from build123d import *

# Parameters (mm, degrees)
SKETCH1_R           = 5
BOSS_EXTRUDE1_DEPTH = 25
SKETCH2_R           = 7.5
BOSS_EXTRUDE2_DEPTH = 8
SKETCH3_R           = 5
BOSS_EXTRUDE3_DEPTH = 30
SKETCH4_R           = 7.5
BOSS_EXTRUDE4_DEPTH = 17
CHAMFER1_SIZE       = 1
CHAMFER2_SIZE       = 0.5


with BuildPart() as part:
    # Sketch1 → Boss-Extrude1 (new body)
    with BuildSketch(Plane.XY):
        Circle(SKETCH1_R)
    extrude(amount=BOSS_EXTRUDE1_DEPTH)

    # Sketch2 → Boss-Extrude2 (add)
    with BuildSketch(Plane.XY.offset(25)):
        Circle(SKETCH2_R)
    extrude(amount=BOSS_EXTRUDE2_DEPTH)

    # Sketch3 → Boss-Extrude3 (add)
    with BuildSketch(Plane.XY.offset(33)):
        Circle(SKETCH3_R)
    extrude(amount=BOSS_EXTRUDE3_DEPTH)

    # Sketch4 → Boss-Extrude4 (add)
    with BuildSketch(Plane.XY.offset(33)):
        Circle(SKETCH4_R)
    extrude(amount=BOSS_EXTRUDE4_DEPTH)

    # Chamfer1
    chamfer1_edges = [part.edges().sort_by_distance(p)[0] for p in [
        (-7.5, 0, 50),
    ]]
    chamfer(chamfer1_edges, length=CHAMFER1_SIZE)

    # Chamfer2
    chamfer2_edges = [part.edges().sort_by_distance(p)[0] for p in [
        (-5, 0, 63),
    ]]
    chamfer(chamfer2_edges, length=CHAMFER2_SIZE)


solid = part.part
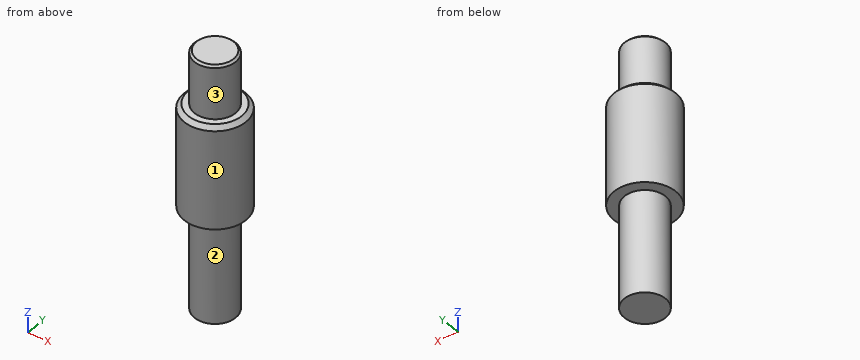
Can you work these out from the model? Positions are in its coordinate system, mm. Face numbers are marked on the shaded views. A direction names the side the tool comes from. Coordinates: 2 decimals unless noted, no trailing zeros. Write each loop counter-clockwise with the first axis right and the second up, starting at its lowest first coordinate (ties: lowest second). Pieces come first, ordered by that corner, then holes. Notation, with made-up numbers: (-39.75, 35.25) -> (-19.75, 35.25) arc R25 ccw to (-19.75, 56.25) -> close; hole circle Ø7 at (85, 18). An arc over 180 degrees is marked (long way). Write each question's results on one line, items separated by ' | '. Start each with the question number.
Item 1: Please list where these lines run through material, in increasing order: probe 1 along Z at (x, y) = (-5.25, -3); probe 2 along X at (y, z) = (5.75, 43); probe 3 along X at (y, z) = (6.5, 33.5).
Item 2: If we section it at D-D, the plane z = 24: Write out the boundary of the cut face in (x, y), and give its area (3 significant figures).
Item 3: I'm going to push flat-ended pins straight in: P1, Ø2, axis at y = 3, z = 19.5, coming from the -X side; P2, Ø6, axis at x = -1, z = 47.5, coming from the -Y side; P3, Ø4, axis at y = 2.5, z = 36.5, coming from the +X side; P4, Ø3, axis at x = 4.5, z = 9, coming from the +Y side. Where does each tip first touch, or does it pass through?
Item 4: If we section it at C-C, the plane z = 34: Write out the boundary of the cut face in (x, y).
Item 5: If we section it at A-A, the plane y = 0: Write out the boundary of the cut face in (x, z), and give its area (3 significant figures).
Item 6: On a 3-axis mill with a long thin cutter (end or side, diameter ignored), from which of +Z, -Z, +X, -X, +Y, -Y can I reach the whole of each face in a straight line? I mean the marked faces 1, 2 and 3. Say none if no direction works.
Answer block:
1) probe 1: 25 to 50 | probe 2: -4.82 to 4.82 | probe 3: -3.74 to 3.74
2) outline: circle Ø10 at (0, 0) | area: 78.5 mm²
3) P1: x = -4.58 | P2: y = -7.5 | P3: x = 7.48 | P4: y = 4
4) outline: circle Ø15 at (0, 0)
5) outline: (-7.5, 25) -> (-5, 25) -> (-5, 0) -> (5, 0) -> (5, 25) -> (7.5, 25) -> (7.5, 49) -> (6.5, 50) -> (5, 50) -> (5, 62.5) -> (4.5, 63) -> (-4.5, 63) -> (-5, 62.5) -> (-5, 50) -> (-6.5, 50) -> (-7.5, 49) -> close | area: 754 mm²
6) face 1: +Z, -Z | face 2: -Z | face 3: +Z
